Check sheet for the drawn part. Datum: minimum x, y, z corner. Units: mm. A direction names the side the tool comes from. Coordinates: 2 decimals unless noted, no trailing zeros. Write each loop counter-clockwise with the first axis right and the second up, starting at its lowest first coordinate (ties: lowest second). Pieces come first, ordered by that corner, then holes. Notation, with made-up numbers: (-22, 45) -> (-4, 45) arc R9 cw to (-4, 55) -> close; hole circle Ø8 at (-19, 52.25). An arc over 180 degrees is marked (long way). Answer in a Markdown table with one row per item.
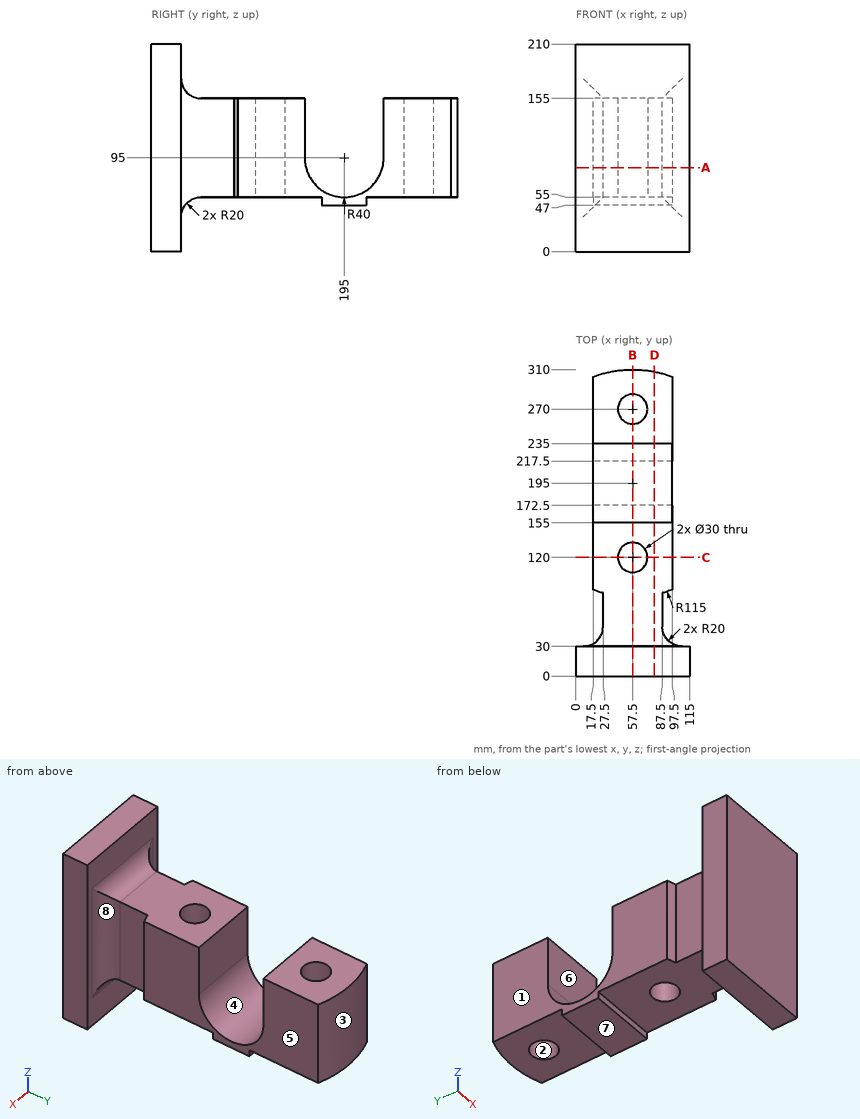
1. Go/stop test with flat-tipped pins: pin 1 (1 mm diameter, centred on x = 78.5, y = 37.5, fed in from +Z); pin 2 (17 mm diameter, centred on y = 63.5, z = 106, fed in from -X); pin 3 (1.5 mm diameter, centred on x = 80, y = 235, fed in from -Z). Record where each tip stops, or that it passes through.
Findings below:
| item | result |
|---|---|
| pin 1 | stops at z = 159.8 |
| pin 2 | stops at x = 27.5 |
| pin 3 | stops at z = 55 |
2. Sectioned sample at D-D, the plane x = 79.5. Record the cut outline in (y, z), and give its area (3 significant figures).
Findings below:
| item | result |
|---|---|
| outline | (0, 0) -> (30, 0) -> (30, 35) arc R20 cw to (50, 55) -> (172.5, 55) -> (172.5, 47) -> (217.5, 47) -> (217.5, 55) -> (307.88, 55) -> (307.88, 155) -> (235, 155) -> (235, 95) arc R40 cw to (155, 95) -> (155, 155) -> (50, 155) arc R20 cw to (30, 175) -> (30, 210) -> (0, 210) -> close |
| area | 27,300 mm² |
3. Sectioned sample at B-B, the plane x = 57.5. Record the cut outline in (y, z).
Findings below:
| item | result |
|---|---|
| outline | (0, 0) -> (30, 0) -> (30, 35) arc R20 cw to (50, 55) -> (105, 55) -> (105, 155) -> (50, 155) arc R20 cw to (30, 175) -> (30, 210) -> (0, 210) -> close; (135, 55) -> (172.5, 55) -> (172.5, 47) -> (217.5, 47) -> (217.5, 55) -> (255, 55) -> (255, 155) -> (235, 155) -> (235, 95) arc R40 cw to (155, 95) -> (155, 155) -> (135, 155) -> close; (285, 55) -> (310, 55) -> (310, 155) -> (285, 155) -> close |
4. Access from +Z, -Z, +X, -X, +Y, -Y to the whole of each face (thin tool, end or side, straight path). Record for the marked faces 5, 6, 7 and 8.
Findings below:
| item | result |
|---|---|
| face 5 | +Z, -Z, +X, +Y |
| face 6 | +Z, +X, -X |
| face 7 | -Z, +X, -X, +Y |
| face 8 | +Z, -Z, +X |
5. Release check for a two-part mould opening along Y. For the marked faces 1, 2, 3 and 4 record: released by +Y, released by -Y, zero draft, split by the parting line, or undercut.
Findings below:
| item | result |
|---|---|
| face 1 | zero draft |
| face 2 | undercut |
| face 3 | released by +Y |
| face 4 | undercut |
6. Sectioned sample at C-C, the plane y = 120. Record the cut outline in (x, z).
Findings below:
| item | result |
|---|---|
| outline | (17.5, 55) -> (42.5, 55) -> (42.5, 155) -> (17.5, 155) -> close; (72.5, 55) -> (97.5, 55) -> (97.5, 155) -> (72.5, 155) -> close |
7. Material ranges on probe 1 along Y at (x, z) = (57.5, 106); probe 2 along X at (y, z) = (120, 108); probe 3 along Y at (x, z) = (57.5, 88.5), recorded low to high. Write a range as from..to.
Findings below:
| item | result |
|---|---|
| probe 1 | y = 0..105, 135..155, 235..255, 285..310 |
| probe 2 | x = 17.5..42.5, 72.5..97.5 |
| probe 3 | y = 0..105, 135..155.53, 234.47..255, 285..310 |
8. Sectioned sample at A-A, the plane z = 85. Record the cut outline in (x, y).
Findings below:
| item | result |
|---|---|
| outline | (0, 0) -> (115, 0) -> (115, 30) -> (107.5, 30) arc R20 cw to (87.5, 50) -> (87.5, 83.98) arc R115 ccw to (97.5, 87.18) -> (97.5, 156.27) -> (17.5, 156.27) -> (17.5, 87.18) arc R115 ccw to (27.5, 83.98) -> (27.5, 50) arc R20 cw to (7.5, 30) -> (0, 30) -> close; (17.5, 233.73) -> (97.5, 233.73) -> (97.5, 302.82) arc R115 ccw to (17.5, 302.82) -> close; hole circle Ø30 at (57.5, 120); hole circle Ø30 at (57.5, 270) |
